from build123d import *

# Parameters (mm, degrees)
SKETCH_1_W                = 50
SKETCH_1_H                = 60
EXTRUDE_1_DEPTH           = 5
HOLE_WIZARD_1_D           = 4.5
HOLE_WIZARD_1_CBORE_D     = 8
HOLE_WIZARD_1_CBORE_DEPTH = 4.6
M8X1_0_1_D                = 7
SKETCH_8_W                = 30
SKETCH_8_H                = 70
EXTRUDE_2_DEPTH           = 10
CHAMFER_1_SIZE            = 1
FILLET_1_R                = 5
HOLE_WIZARD_M4_1_D        = 3.3
HOLE_WIZARD_M4_1_DEPTH    = 10.1
HOLE_WIZARD_M4_1_TIP      = 0.991420021


with BuildPart() as part:
    # 草图1 → 凸台-拉伸1 (new, symmetric)
    with BuildSketch(Plane(origin=(0, 0, 0), x_dir=(1, 0, 0), z_dir=(0, 1, 0))):
        Rectangle(SKETCH_1_W, SKETCH_1_H)
    extrude(amount=EXTRUDE_1_DEPTH, both=True)

    # 打孔尺寸(%根据)内六角圆柱头螺钉的类型1 (through all)
    with Locations(Plane(origin=(0, 5, 0), x_dir=(1, 0, 0), z_dir=(0, 1, 0))):
        with Locations((13, -24), (13, 2), (-13, 2), (-13, -24)):
            CounterBoreHole(HOLE_WIZARD_1_D / 2, HOLE_WIZARD_1_CBORE_D / 2, HOLE_WIZARD_1_CBORE_DEPTH)

    # M8x1.0 螺纹孔1 (through all)
    with Locations(Plane(origin=(0, 5, 0), x_dir=(1, 0, 0), z_dir=(0, 1, 0))):
        with Locations((-14, 14), (14, 14)):
            Hole(M8X1_0_1_D / 2)

    # 草图8 → 凸台-拉伸2 (add)
    with BuildSketch(Plane(origin=(0, 5, 0), x_dir=(1, 0, 0), z_dir=(0, 1, 0))):
        with Locations((0, 65)):
            Rectangle(SKETCH_8_W, SKETCH_8_H)
    extrude(amount=-EXTRUDE_2_DEPTH)

    # 倒角1
    chamfer_1_edges = [part.edges().sort_by_distance(p)[0] for p in [
        (25, 0, 30),
        (-25, 0, 30),
        (-25, 0, -30),
        (25, 0, -30),
    ]]
    chamfer(chamfer_1_edges, length=CHAMFER_1_SIZE)

    # 圆角1
    fillet_1_edges = [part.edges().sort_by_distance(p)[0] for p in [
        (-15, 0, -30),
        (15, 0, -30),
    ]]
    fillet(fillet_1_edges, radius=FILLET_1_R)

    # M4 螺纹孔1
    with Locations(Plane(origin=(0, 0, -100), x_dir=(-1, 0, 0), z_dir=(0, 0, -1))):
        with Locations((10, 0), (-10, 0)):
            Hole(HOLE_WIZARD_M4_1_D / 2, depth=HOLE_WIZARD_M4_1_DEPTH)
            with Locations((0, 0, -(HOLE_WIZARD_M4_1_DEPTH + HOLE_WIZARD_M4_1_TIP / 2))):  # 118° drill point
                Cone(0, HOLE_WIZARD_M4_1_D / 2, HOLE_WIZARD_M4_1_TIP, mode=Mode.SUBTRACT)


solid = part.part
The model under review builds one solid part; all positions refer to its coordinate system, in mm. A direction names the side the tool comes from. Give positions to 0.01 mm unless a question says otherwise; leave off trailing zeros. Loops run counter-clockwise (first coordinate to the right, second up) from the corner with the lowest first, then second, coordinate; pieces in that order, holes last. Notation, with made-up numbers: (36, 79.5) -> (77, 79.5) arc R25 ccw to (77, 99.5) -> close; hole circle Ø8 at (-33, -27.5). An arc over 180 degrees is marked (long way). Put each result on its own line as item: value. Start each with the question number.
1. Mouldability with a two-part tool opening along Z and no side actions: class faces 1 (the face through (0, -5, -21)), 2 (the face through (16, 0, -32)), 3 (the face through (15, 0.4, 26)) as released by +Z, released by -Z, zero draft, split by the parting line, or undercut.
2. Wall thickness on probe 1 along X at (y, z) = (-1.95, 24); probe 2 along X at (y, z) = (2.85, 24); probe 3 along Z at (x, y) = (-13, 3.25): over which ranges is each line inside the solid? List them lowest first.
3. We need section B-B on z = 24. State the section outline as (x, y) points, then the cut area to 3 significant figures.
4. We need section A-A on y = -3.5. State the section outline as (x, z) points, then the cut area to 3 significant figures.
5. Clearance check with flat-ended pins moving along their axes: P1, Ø3, axis at x = 23, y = 2, coming from the -Z side; P2, Ø6, axis at x = 13, z = 24, coming from the +Y side; P3, Ø1.5, axis at x = -18, y = 0.5, coming from the -Z side. State where each tip first meets the part, or that it passes through.
6. We need section C-C on x = -13. State the section outline as (y, z) points.
7. For faces 4 (the face through (-22, 0, -30)), 5 (the face through (-16.2, 2.7, 0.4)), 6 (the face through (-8.476, -0.632, -94.879)), list the 3-axis set-ups (+Z, -Z, +X, -X, +Y, -Y) from which the entire face can be reached by the end or side of a thin tool; tool diameter is ignored.
8. We need section D-D on z = -14. State the section outline as (x, y) points, then the cut area to 3 significant figures.
Determined:
1. face 1: zero draft
1. face 2: released by -Z
1. face 3: undercut
2. probe 1: -25 to -15.25, -10.75 to 10.75, 15.25 to 25
2. probe 2: -25 to -17, -9 to 9, 17 to 25
2. probe 3: -100 to -17.35, -10.65 to -6, 2 to 20, 28 to 30
3. outline: (-25, -5) -> (-15.25, -5) -> (-15.25, 0.4) -> (-17, 0.4) -> (-17, 5) -> (-25, 5) -> close; (-10.75, -5) -> (10.75, -5) -> (10.75, 0.4) -> (9, 0.4) -> (9, 5) -> (-9, 5) -> (-9, 0.4) -> (-10.75, 0.4) -> close; (15.25, -5) -> (25, -5) -> (25, 5) -> (17, 5) -> (17, 0.4) -> (15.25, 0.4) -> close
3. area: 378 mm^2
4. outline: (-25, -29) -> (-24, -30) -> (-20, -30) arc R5 cw to (-15, -35) -> (-15, -100) -> (15, -100) -> (15, -35) arc R5 cw to (20, -30) -> (24, -30) -> (25, -29) -> (25, 29) -> (24, 30) -> (-24, 30) -> (-25, 29) -> close; hole circle Ø7 at (-14, -14); hole circle Ø4.5 at (-13, -2); hole circle Ø4.5 at (-13, 24); hole circle Ø7 at (14, -14); hole circle Ø4.5 at (13, -2); hole circle Ø4.5 at (13, 24)
4. area: 4,970 mm^2
5. P1: z = -30
5. P2: y = 0.4
5. P3: z = -30.82
6. outline: (-5, -100) -> (5, -100) -> (5, -17.35) -> (-5, -17.35) -> close; (-5, -10.65) -> (5, -10.65) -> (5, -6) -> (0.4, -6) -> (0.4, -4.25) -> (-5, -4.25) -> close; (-5, 0.25) -> (0.4, 0.25) -> (0.4, 2) -> (5, 2) -> (5, 20) -> (0.4, 20) -> (0.4, 21.75) -> (-5, 21.75) -> close; (-5, 26.25) -> (0.4, 26.25) -> (0.4, 28) -> (5, 28) -> (5, 30) -> (-5, 30) -> close
7. face 4: -Z, -X, +Y, -Y
7. face 5: +Y
7. face 6: -Z
8. outline: (-25, -5) -> (-17.5, -5) -> (-17.5, 5) -> (-25, 5) -> close; (-10.5, -5) -> (10.5, -5) -> (10.5, 5) -> (-10.5, 5) -> close; (17.5, -5) -> (25, -5) -> (25, 5) -> (17.5, 5) -> close
8. area: 360 mm^2
